from build123d import *

# Parameters (mm, degrees)
EXTRUDE_1_DEPTH        = 12
HOLE_WIZARD_M5_1_D     = 4.2
HOLE_WIZARD_M5_1_DEPTH = 10
HOLE_WIZARD_M5_1_TIP   = 1.2618073
HOLE_WIZARD_M5_2_D     = 4.2
HOLE_WIZARD_M5_2_DEPTH = 10
HOLE_WIZARD_M5_2_TIP   = 1.2618073


with BuildPart() as part:
    # 草图1 → 凸台-拉伸1 (new body)
    with BuildSketch(Plane.XY):
        Polygon((-30.106749708, 4.118589161), (-40.106749708, 4.118589161), (-40.106749708, 34.118589161), (14.893250292, 34.118589161), (14.893250292, 24.118589161), align=None)
    extrude(amount=EXTRUDE_1_DEPTH)

    # M5 螺纹孔1
    with Locations(Plane(origin=(-24.106749708, 34.118589161, 6), x_dir=(0, 0, 1), z_dir=(0, 1, 0))):
        with Locations((0, 0), (0, 30)):
            Hole(HOLE_WIZARD_M5_1_D / 2, depth=HOLE_WIZARD_M5_1_DEPTH)
            with Locations((0, 0, -(HOLE_WIZARD_M5_1_DEPTH + HOLE_WIZARD_M5_1_TIP / 2))):  # 118° drill point
                Cone(0, HOLE_WIZARD_M5_1_D / 2, HOLE_WIZARD_M5_1_TIP, mode=Mode.SUBTRACT)

    # M5 螺纹孔2
    with Locations(Plane(origin=(-40.106749708, 9.118589161, 6), x_dir=(0, 0, -1), z_dir=(-1, 0, 0))):
        with Locations((0, 0), (0, -20)):
            Hole(HOLE_WIZARD_M5_2_D / 2, depth=HOLE_WIZARD_M5_2_DEPTH)
            with Locations((0, 0, -(HOLE_WIZARD_M5_2_DEPTH + HOLE_WIZARD_M5_2_TIP / 2))):  # 118° drill point
                Cone(0, HOLE_WIZARD_M5_2_D / 2, HOLE_WIZARD_M5_2_TIP, mode=Mode.SUBTRACT)


solid = part.part
Could you check a few things on this model? Use its own coordinates, in mm. A direction names the side the tool comes from. Round coordinates to 2 decimals unless told otherwise and drop trailing zeros. Order: outer loops, then holes, each group sorted by start corner. A loop starts at its lowest first (then second) coordinate and runs counter-clockwise, first axis right, second up.
(1) Imagine slicing it at A-A (z = 2.5). Write out the boundary of the cut face in (x, y), plus the area to 3 significant figures.
Response values:
outline: (-40.11, 4.12) - (-30.11, 4.12) - (14.89, 24.12) - (14.89, 34.12) - (-40.11, 34.12) - close
area: 1,200 mm2
(2) If we mould it in two halves opening along Z, with no side actions, what happens to faces 4 (the flat face through (-7.29, 14.26, 5.92)), 5 (the flat face through (-18, 23, 0)), 6 (the cylindrical face through (7.975, 29.049, 6.273))? For each: released by +Z, released by -Z, zero draft, split by the parting line, or undercut.
Response values:
face 4: zero draft
face 5: released by -Z
face 6: undercut
(3) Imagine slicing it at B-B (x = -3.5). Write out the boundary of the cut face in (y, z).
Response values:
outline: (15.94, 0) - (34.12, 0) - (34.12, 12) - (15.94, 12) - close
(4) Which directions (+Z, -Z, +X, -X, +Y, -Y) give clear straight access to the entire face, cutting with the end or side of a thin tool? Please do faces 1 (the cylindrical face through (-26.157, 29.049, 6.455)), 2 (the flat face through (-13, 34.119, 6)), 3 (the cylindrical face through (-35.037, 11.169, 5.545)).
Response values:
face 1: +Y
face 2: +Z, -Z, +X, -X, +Y
face 3: -X
(5) I'm going to push flat-ended pins straight in: pin 1 (6.5 mm diameter, centred on x = -24.11, z = 6, fed in from -Y); pin 2 (6.5 mm diameter, centred on y = 9.12, z = 6, fed in from +X); pin 3 (2.5 mm diameter, centred on x = 5.89, z = 6, fed in from +Y). Where does each tip first touch, or does it pass through?
Response values:
pin 1: stops at y = 5.34
pin 2: stops at x = -11.54
pin 3: stops at y = 23.61
(6) Imagine slicing it at C-C (y = 14). Write out the boundary of the cut face in (x, z).
Response values:
outline: (-40.11, 0) - (-7.87, 0) - (-7.87, 12) - (-40.11, 12) - close
(7) Please list where these lines run through material, in increasing order: line 1 along X through (y, z) = (32, 6); line 2 along Y through (x, z) = (-36.5, 6); line 3 along X through (y, z) = (27.5, 6).
Response values:
line 1: x = -40.11 to -26.21, -22.01 to 3.79, 7.99 to 14.89
line 2: y = 4.12 to 7.02, 11.22 to 27.02, 31.22 to 34.12
line 3: x = -29.82 to -26.21, -22.01 to 3.79, 7.99 to 14.89
